from build123d import *

# Parameters (mm, degrees)
SKETCH1_R           = 15
BOSS_EXTRUDE1_DEPTH = 10
SKETCH2_R           = 7.5
BOSS_EXTRUDE2_DEPTH = 10
SKETCH3_R           = 4
BOSS_EXTRUDE3_DEPTH = 40
SKETCH4_R           = 5
BOSS_EXTRUDE4_DEPTH = 10
CHAMFER1_SIZE       = 0.5


with BuildPart() as part:
    # Sketch1 → Boss-Extrude1 (new body)
    with BuildSketch(Plane.XY):
        Circle(SKETCH1_R)
    extrude(amount=BOSS_EXTRUDE1_DEPTH)

    # Sketch2 → Boss-Extrude2 (add)
    with BuildSketch(Plane.XY.offset(10)):
        Circle(SKETCH2_R)
    extrude(amount=BOSS_EXTRUDE2_DEPTH)

    # Sketch3 → Boss-Extrude3 (add)
    with BuildSketch(Plane.XY.offset(20)):
        Circle(SKETCH3_R)
    extrude(amount=BOSS_EXTRUDE3_DEPTH)

    # Sketch4 → Boss-Extrude4 (add)
    with BuildSketch(Plane.XY.offset(20)):
        Circle(SKETCH4_R)
    extrude(amount=BOSS_EXTRUDE4_DEPTH)

    # Chamfer1
    chamfer1_edges = [part.edges().sort_by_distance(p)[0] for p in [
        (-4, 0, 60),
        (-5, 0, 30),
        (-15, 0, 0),
        (-15, 0, 10),
        (-7.5, 0, 20),
    ]]
    chamfer(chamfer1_edges, length=CHAMFER1_SIZE)


solid = part.part
Read the model definition and answer for the solid it produces. Units are mm, in the model's axes. A direction names the side the tool comes from. Coordinates: 2 decimals unless noted, no trailing zeros. Loops run counter-clockwise (first coordinate to the right, second up) from the corner with the lowest first, then second, coordinate; pieces in that order, holes last.
Q1. Each of these flat-tipped pins is pushed along its axis until it touches: pin 1 Ø4 at (y, z) = (3, 36.5) entering from -X; pin 2 Ø6 at (x, z) = (2.5, 51) entering from +Y; pin 3 Ø8 at (y, z) = (7.5, 11.5) entering from +X. Where does it stop, or does it pass through?
Q2. The part is cut by section C-C on z = 32. Write down the section's boundary in (x, y).
Q3. The part is cut by section B-B on z = 18.5. Write down the section's boundary in (x, y).
Q4. Consider probe 1 along Z at (x, y) = (7.5, 2); probe 2 along Z at (x, y) = (-0.25, -7); probe 3 along Y at (x, z) = (0, 6). Determine where each line is inside the solid, lowest interval first.
Q5. Which of the six approach directions +Z, -Z, +X, -X, +Y, -Y give full straight-line access (tool end or side, diameter ignored) to faces 1 (the face through (-14.985, 0.66, 4.937)), 2 (the face through (-3, -3, 30))?
Q6. The part is cut by section A-A on x = 0. Write down the section's boundary in (y, z), and give its area (3 significant figures).
Results below:
1. pin 1: stops at x = -3.87
1. pin 2: stops at y = 4
1. pin 3: stops at x = 14.45
2. outline: circle Ø8 at (0, 0)
3. outline: circle Ø15 at (0, 0)
4. probe 1: z = 0 to 10
4. probe 2: z = 0 to 20
4. probe 3: y = -15 to 15
5. face 1: +Z, -Z
5. face 2: +Z
6. outline: (-15, 0.5) - (-14.5, 0) - (14.5, 0) - (15, 0.5) - (15, 9.5) - (14.5, 10) - (7.5, 10) - (7.5, 19.5) - (7, 20) - (5, 20) - (5, 29.5) - (4.5, 30) - (4, 30) - (4, 59.5) - (3.5, 60) - (-3.5, 60) - (-4, 59.5) - (-4, 30) - (-4.5, 30) - (-5, 29.5) - (-5, 20) - (-7, 20) - (-7.5, 19.5) - (-7.5, 10) - (-14.5, 10) - (-15, 9.5) - close
6. area: 789 mm2
